from build123d import *

# Parameters (mm, degrees)
BOSS_EXTRUDE1_DEPTH = 10
SKETCH3_R           = 8
BOSS_EXTRUDE2_DEPTH = 5
SKETCH4_R           = 6
BOSS_EXTRUDE3_DEPTH = 15
CHAMFER1_SIZE       = 1


with BuildPart() as part:
    # Sketch1 → Revolve2 (revolve)
    with BuildSketch(Plane.XY, mode=Mode.PRIVATE) as revolve2_sk:
        with BuildLine():
            Line((-2, 0), (-2, 27))
            Line((-2, 27), (-4, 27))
            Line((-4, 27), (-4, 30))
            Line((-4, 30), (-8, 30))
            Line((-8, 30), (-8, 8.392398037))
            Line((-8, 8.392398037), (-6.75, 8.392398037))
            ThreePointArc((-6.75, 8.392398037), (-6.244894811, 3.375866985), (-2.5, 0))
            Line((-2.5, 0), (-2, 0))
        make_face()
    revolve(revolve2_sk.sketch.rotate(Axis((0, 0, 0), (0, 1, 0)), 270), axis=Axis((0, 0, 0), (0, 1, 0)))

    # Sketch2 → Boss-Extrude1 (add)
    with BuildSketch(Plane(origin=(0, 30, 0), x_dir=(1, 0, 0), z_dir=(0, 1, 0))):
        with BuildLine():
            Line((-4, 6.92820323), (-4, 4.472135955))
            ThreePointArc((-4, 4.472135955), (0, -6), (4, 4.472135955))
            Line((4, 4.472135955), (4, 6.92820323))
            ThreePointArc((4, 6.92820323), (0, -8), (-4, 6.92820323))
        make_face()
    extrude(amount=BOSS_EXTRUDE1_DEPTH)

    # Sketch3 → Boss-Extrude2 (add)
    with BuildSketch(Plane(origin=(0, 40, 0), x_dir=(1, 0, 0), z_dir=(0, 1, 0))):
        with Locations(Location((0, 0, 0), (0, 0, 90))):
            Circle(SKETCH3_R)
    extrude(amount=BOSS_EXTRUDE2_DEPTH)

    # Sketch4 → Boss-Extrude3 (add)
    with BuildSketch(Plane(origin=(0, 45, 0), x_dir=(1, 0, 0), z_dir=(0, 1, 0))):
        with Locations(Location((0, 0, 0), (0, 0, 270))):
            Circle(SKETCH4_R)
    extrude(amount=BOSS_EXTRUDE3_DEPTH)

    # Chamfer1
    chamfer1_edges = [part.edges().sort_by_distance(p)[0] for p in [
        (0, 45, 8),
        (0, 60, -6),
    ]]
    chamfer(chamfer1_edges, length=CHAMFER1_SIZE)


solid = part.part
Build history of the part. All positions in model axes, mm. A direction names the side the tool comes from. Round coordinates to 2 decimals unless told otherwise and drop trailing zeros. Order: outer loops, then holes, each group sorted by start corner. A loop starts at its lowest first (then second) coordinate and runs counter-clockwise, first axis right, second up. Notation, with made-up numbers: M 44.25,-11.5 L 99.25,-11.5 A31 ccw 99.25,26.5 Z; hole C 47.5,59.5 d11. An arc over 180 degrees is marked long. Use CSV: the item, a comma, the result in double quotes. Start each with the question number.
(1) Cut at A-A on x = 0. List the corners of the cut face in (y, z), then the cut area to 3 significant figures.
(2) Tool access for faces 4 (the face through (0, 40, -1)), 5 (the face through (-2, 0, 1)), 6 (the face through (4, 35, -6)), 7 (the face through (1.802, 51.902, 5.723)): list every direction of +Z, -Z, +X, -X, +Y, -Y with a clear straight run to the whole face (end or side of a thin tool).
(3) Cut at B-B on z = 0. List the corners of the cut face in (x, y), then the cut area to 3 significant figures.
(4) Flat gauge pins, fed straight in: P1, Ø2.5, axis at y = 34, z = -5.5, coming from the -X side; P2, Ø0.7, axis at y = 33.5, z = -5, coming from the +X side; P3, Ø6, axis at y = 16.5, z = 3.5, coming from the -X side. Where does each tip first touch, or does it go through?
(5) Cut at C-C on y = 10. List the corners of the cut face in (x, z), then the cut area to 3 significant figures.
(6) Mould opens along Y. For faces 1 (the face through (0, 60, 0)), 2 (the face through (2, 14, 0)), 3 (the face through (-4, 35, -6)) say: +Y half, -Y half, draft (parallel to the pull), parting line (faces both ways), or undercut.
(7) Drill centre lines: probe 1 along X at (y, z) = (20.5, 0); probe 2 along X at (y, z) = (28.9, 0); probe 3 along Z at (x, y) = (0, 32.75). Where is each one in solid material? Low to high.
Findings:
1,outline,"M 0,-2.5 A7 ccw 8.39,-6.75 L 8.39,-8 L 30,-8 L 30,-4 L 27,-4 L 27,-2 L 0,-2 Z; M 0,2 L 27,2 L 27,4 L 30,4 L 30,6 L 40,6 L 40,-8 L 44,-8 L 45,-7 L 45,-6 L 59,-6 L 60,-5 L 60,5 L 59,6 L 45,6 L 45,7 L 44,8 L 8.39,8 L 8.39,6.75 A7 ccw 0,2.5 Z"
1,area,"593 mm^2"
2,face 4,"none"
2,face 5,"+Z, -Z, +X, -X, -Y"
2,face 6,"-Z"
2,face 7,"+Y"
3,outline,"M -8,8.39 L -6.75,8.39 A7 ccw -2.5,0 L -2,0 L -2,27 L -4,27 L -4,30 L -6,30 L -6,40 L 6,40 L 6,30 L 4,30 L 4,27 L 2,27 L 2,0 L 2.5,0 A7 ccw 6.75,8.39 L 8,8.39 L 8,44 L 7,45 L 6,45 L 6,59 L 5,60 L -5,60 L -6,59 L -6,45 L -7,45 L -8,44 Z"
3,area,"613 mm^2"
4,P1,"stops at x = -6.78"
4,P2,"stops at x = 6.51"
4,P3,"stops at x = -7.98"
5,outline,"C 0,0 d16; hole C 0,0 d4"
5,area,"188 mm^2"
6,face 1,"+Y half"
6,face 2,"draft"
6,face 3,"undercut"
7,probe 1,"x = -8 to -2, 2 to 8"
7,probe 2,"x = -8 to -4, 4 to 8"
7,probe 3,"z = 6 to 8"
